from build123d import *

# Parameters (mm, degrees)
FILLET_1_R          = 0.5
CHAMFER_1_SIZE      = 1.732050808
CHAMFER_1_SIZE2     = 1
SKETCH_2_R          = 1.07
CUT_EXTRUDE_1_DEPTH = 500


with BuildPart() as part:
    # 草图1 → Revolve 730 (revolve)
    with BuildSketch(Plane.XY, mode=Mode.PRIVATE) as revolve_730_sk:
        with BuildLine():
            Line((0, 0), (28, 0))
            Line((28, 0), (28, 3))
            Line((28, 3), (2, 3))
            Line((2, 3), (2, 4))
            ThreePointArc((2, 4), (1, 5), (0, 4))
            Line((0, 4), (0, 0))
        make_face()
    revolve(revolve_730_sk.sketch.rotate(Axis((0, 0, 0), (1, 0, 0)), 90), axis=Axis((0, 0, 0), (1, 0, 0)))

    # 圆角1
    fillet_1_edges = [part.edges().sort_by_distance(p)[0] for p in [
        (2, 0, -3),
    ]]
    fillet(fillet_1_edges, radius=FILLET_1_R)

    # 倒角1
    chamfer_1_edges = [part.edges().sort_by_distance(p)[0] for p in [
        (28, 0, -3),
    ]]
    chamfer_1_side = [part.faces().sort_by_distance(p)[0] for p in [
        (15.25, 0, -3),
    ]]
    chamfer(chamfer_1_edges, length=CHAMFER_1_SIZE, length2=CHAMFER_1_SIZE2, reference=chamfer_1_side[0])

    # 草图2 → 切除-拉伸1 (cut, symmetric)
    with BuildSketch(Plane(origin=(0, 0, 0), x_dir=(1, 0, 0), z_dir=(0, 1, 0))):
        with Locations(Location((25, 0, 0), (0, 0, 270))):
            Circle(SKETCH_2_R)
    extrude(amount=CUT_EXTRUDE_1_DEPTH, both=True, mode=Mode.SUBTRACT)


solid = part.part
Work out the finished part from the listing and answer in its coordinate system (mm). Round coordinates to 2 decimals unless told otherwise and drop trailing zeros. Write each loop counter-clockwise with the first axis right and the second up, starting at its lowest first coordinate (ties: lowest second). Pieces come first, ordered by that corner, then holes. Notation, with made-up numbers: (85, -17) -> (137, -17) arc R20 ccw to (137, 13) -> close; hole circle Ø6 at (20, 33.25). An arc over 180 degrees is marked (long way). Answer as CSV lines item,"result". Start each with the question number.
(1) Each of these flat-tipped pins is pushed along its axis until it touches: pin 1 (1 mm diameter, centred on x = 11, y = -1.5, fed in from -Z); pin 2 (5 mm diameter, centred on x = 24.5, y = -1, fed in from +Z); pin 3 (3 mm diameter, centred on x = 25, z = 0, fed in from -Y). Where does it stop, or does it pass through?
(2) The part is cut by section A-A, the plane z = 0. Give the vertices of the cut face in (x, y), then the cut area to 3 significant figures.
(3) The part is cut by section B-B, the plane y = 0. Give the vertices of the cut face in (x, z), then the cut area to 3 significant figures.
(4) Find the intervals of material crossed by probe 1 along X at (y, z) = (-1.5, 0); probe 2 along X at (y, z) = (0.5, 0.5); probe 3 along X at (y, z) = (-3.5, 1.25), in increasing order.
(5) The mould has two halves that part along X. Classify faces 1 (the flat face through (28, 0, 0)), 2 (the flat face through (0, 0, 0)), 3 (the cylindrical face through (23.955, 0.042, -0.232)): +X half, -X half, draft (parallel to the pull), parting line (faces both ways), or undercut.
(6) The part is cut by section C-C, the plane x = 25. Give the vertices of the cut face in (y, z), then the cut area to 3 significant figures.
(7) The part is cut by section D-D, the plane x = 6.25. Give the vertices of the cut face in (y, z), then the cut area to 3 significant figures.
Output values:
1,pin 1,"stops at z = -2.83"
1,pin 2,"stops at z = 3"
1,pin 3,"stops at y = -3"
2,outline,"(0, -4) arc R1 ccw to (2, -4) -> (2, -3.5) arc R0.5 cw to (2.5, -3) -> (23.93, -3) -> (23.93, 3) -> (2.5, 3) arc R0.5 cw to (2, 3.5) -> (2, 4) arc R1 ccw to (0, 4) -> close; (26.07, -3) -> (26.27, -3) -> (28, -2) -> (28, 2) -> (26.27, 3) -> (26.07, 3) -> close"
2,area,"161 mm²"
3,outline,"(0, -4) arc R1 ccw to (2, -4) -> (2, -3.5) arc R0.5 cw to (2.5, -3) -> (26.27, -3) -> (28, -2) -> (28, 2) -> (26.27, 3) -> (2.5, 3) arc R0.5 cw to (2, 3.5) -> (2, 4) arc R1 ccw to (0, 4) -> close; hole circle Ø2.14 at (25, 0)"
3,area,"170 mm²"
4,probe 1,"x = 0 to 23.93, 26.07 to 28"
4,probe 2,"x = 0 to 24.05, 25.95 to 28"
4,probe 3,"x = 0 to 2"
5,face 1,"+X half"
5,face 2,"-X half"
5,face 3,"undercut"
6,outline,"(-2.8, -1.07) arc R3 ccw to (2.8, -1.07) -> close; (-2.8, 1.07) -> (2.8, 1.07) arc R3 ccw to start"
6,area,"15.7 mm²"
7,outline,"circle Ø6 at (0, 0)"
7,area,"28.3 mm²"
